Design review of the part built by this model. Coordinates are the model's own, in mm. A direction names the side the tool comes from. Give positions to 0.01 mm unless a question says otherwise; leave off trailing zeros. Loops run counter-clockwise (first coordinate to the right, second up) from the corner with the lowest first, then second, coordinate; pieces in that order, holes last. Notation, with made-up numbers: M 53.5,-11.5 L 75.5,-11.5 A11 cw 75.5,4.5 Z; hole C 52.5,29 d6. An arc over 180 degrees is marked long. Use CSV: the item, a comma, the result in double quotes.
from build123d import *

# Parameters (mm, degrees)
BOSS_EXTRUDE1_DEPTH = 22
SKETCH2_W           = 2.8
SKETCH2_H           = 0.5
BOSS_EXTRUDE2_DEPTH = 17.7
SKETCH3_R           = 1.25
SKETCH3_R_2         = 1.05
CUT_EXTRUDE1_DEPTH  = 1
SKETCH4_R           = 1.35
BOSS_EXTRUDE3_DEPTH = 6


with BuildPart() as part:
    # Sketch1 → Boss-Extrude1 (new body)
    with BuildSketch(Plane.XY):
        with BuildLine():
            Line((1.4, 1.428285686), (1.4, 2))
            Line((1.4, 2), (-1.4, 2))
            Line((-1.4, 2), (-1.4, 1.428285686))
            ThreePointArc((-1.4, 1.428285686), (0, -2), (1.4, 1.428285686))
        make_face()
    extrude(amount=-BOSS_EXTRUDE1_DEPTH)

    # Sketch2 → Boss-Extrude2 (add)
    with BuildSketch(Plane.XY.offset(-22)):
        with Locations((0, 2.25)):
            Rectangle(SKETCH2_W, SKETCH2_H)
    extrude(amount=BOSS_EXTRUDE2_DEPTH)

    # Sketch3 → Cut-Extrude1 (cut)
    with BuildSketch(Plane(origin=(0, 2, 0), x_dir=(1, 0, 0), z_dir=(0, 1, 0))):
        with Locations(Location((0, 2, 0), (0, 0, 270))):
            Circle(SKETCH3_R)
        with Locations(Location((0, 2, 0), (0, 0, 270))):
            Circle(SKETCH3_R_2, mode=Mode.SUBTRACT)
    extrude(amount=-CUT_EXTRUDE1_DEPTH, mode=Mode.SUBTRACT)

    # Sketch4 → Boss-Extrude3 (add)
    with BuildSketch(Plane.XY.offset(-22)):
        Circle(SKETCH4_R)
    extrude(amount=-BOSS_EXTRUDE3_DEPTH)


solid = part.part
(1) We need section A-A on z = -2. State the section outline as (x, y) points.
A:
outline,"M -1.4,1.43 A2 ccw long 1.4,1.43 L 1.4,2 L 1.25,2 L 1.25,1 L 1.05,1 L 1.05,2 L -1.05,2 L -1.05,1 L -1.25,1 L -1.25,2 L -1.4,2 Z"
(2) Machinability: for faces 4 (the flat face through (-1.4, 2, -11)), 5 (the flat face through (0, 2, -2)), 6 (the flat face through (-0.9, 1.3, -22)), which of the approach directions +Z, -Z, +X, -X, +Y, -Y give a long, thin tool a straight path to every point of the face, cutting with its end or side? Answer none if there is none.
A:
face 4,"+Z, -Z, -X, +Y"
face 5,"+Z, +X, -X, +Y"
face 6,"-Z"
(3) Clearance check with flat-ended pins moving along their axes: P1, Ø0.8, axis at x = 0.5, z = -1.5, coming from the +Y side; P2, Ø1.5, axis at x = 1.5, z = -14, coming from the -Y side; P3, Ø0.5, axis at y = 2, z = -8.5, coming from the -X side. State where each tip first meets the part, or that it passes through.
A:
P1,"y = 2"
P2,"y = -1.85"
P3,"x = -1.4"
(4) Wall thickness on line 1 along X through (y, z) = (1.75, -2); line 2 along Y through (x, z) = (-0.05, -22.25); line 3 along Y through (x, z) = (0.1, -18.75): over which ranges is each line inside the solid? List them lowest first. Write a range as [from, to].
A:
line 1,"[-1.4, -1.25], [-1.05, 1.05], [1.25, 1.4]"
line 2,"[-1.35, 1.35]"
line 3,"[-2, 2.5]"
(5) We need section D-D on z = -16.25. State the section outline as (x, y) points.
A:
outline,"M -1.4,1.43 A2 ccw long 1.4,1.43 L 1.4,2.5 L -1.4,2.5 Z"
(6) We need section C-C on y = 0. State the section outline as (x, z) points.
A:
outline,"M -2,-22 L -1.35,-22 L -1.35,-28 L 1.35,-28 L 1.35,-22 L 2,-22 L 2,0 L -2,0 Z"
(7) The part is to be moulded in two halves that separate along X. For faces 1 (the flat face through (1.4, 2, -11)), 2 (the cylindrical face through (0, -2, -11)), 3 (the cylindrical face through (0.05, 1.51, -3.05)), say which applies: released by +X, released by -X, zero draft, split by the parting line, or undercut.
A:
face 1,"released by +X"
face 2,"split by the parting line"
face 3,"undercut"
(8) We need section B-B on x = 0. State the section outline as (y, z) points, then the cut area to 3 significant figures.
A:
outline,"M -2,-22 L -1.35,-22 L -1.35,-28 L 1.35,-28 L 1.35,-22 L 2.5,-22 L 2.5,-4.3 L 2,-4.3 L 2,-3.25 L 1,-3.25 L 1,-3.05 L 2,-3.05 L 2,-0.95 L 1,-0.95 L 1,-0.75 L 2,-0.75 L 2,0 L -2,0 Z"
area,"113 mm²"
